Geometry check sheet. Reference: the model listing, model coordinates, mm. A direction names the side the tool comes from. Round coordinates to 2 decimals unless told otherwise and drop trailing zeros. Write each loop counter-clockwise with the first axis right and the second up, starting at its lowest first coordinate (ties: lowest second). Pieces come first, ordered by that corner, then holes. Notation, with made-up numbers: M -3,10.5 L 30,10.5 A13 ccw 30,34.5 Z; hole C 24,3 d7. An arc over 180 degrees is marked long. Put each result on its own line as item: value. Start each with the question number.
(1) Section check C-C on z = 31. Record the cut outline in (x, y).
(2) Tool access check on faces 1 (the cylindrical face through (-15.88, 54.97, 17.32)), 2 (the cylindrical face through (7.086, 50.465, -17.089)), 3 (the flat face through (19.04, 24, 10.33)). Record the directions out of +Z, -Z, +X, -X, +Y, -Y that give a thin tool (end or side, any length) a straight path to the whole face; none if there is none.
(3) Section check D-D on x = 35.5. Record the cut outline in (y, z).
(4) Gauge pin test, flat ends, axial feed: pin 1 (3 mm diameter, centred on y = 49, z = -12.5, fed in from +X); pin 2 (1 mm diameter, centred on y = 16.5, z = 21.5, fed in from +X); pin 3 (10 mm diameter, centred on x = -16.5, y = 57.5, fed in from +Z); pin 4 (1 mm diameter, centred on x = 21, z = 13, fed in from -Y). Record the tip position at first contact, or that the pin passes through.
(5) Material ranges on probe 1 along X at (y, z) = (49.95, 0); probe 2 along Z at (x, y) = (1, 39.5); probe 3 along X at (y, z) = (38.75, 0), recorded low to high.
from build123d import *


with BuildPart() as part:
    # 草图1 → 旋转1 (revolve)
    with BuildSketch(Plane.XY, mode=Mode.PRIVATE) as revolve_1_sk:
        Polygon((-23.5, 57), (-23.5, 53), (-18.5, 53), (-18.5, 48), (-21.5, 48), (-21.5, 24), (-23.5, 24), (-23.5, 0), (-41.5, 0), (-41.5, 6), (-29.5, 6), (-29.5, 20), (-28.5, 20), (-28.5, 67), (-24.5, 67), (-24.5, 57), align=None)
    revolve(revolve_1_sk.sketch.rotate(Axis((0, 0, 0), (0, 1, 0)), 270), axis=Axis((0, 0, 0), (0, 1, 0)))


solid = part.part
Answers follow:
1. outline: M -27.59,0 L 27.59,0 L 27.59,6 L -27.59,6 Z
2. face 1: +Y
2. face 2: +Y, -Y
2. face 3: -Y
3. outline: M 0,-21.49 L 6,-21.49 L 6,21.49 L 0,21.49 Z
4. pin 1: stops at x = 26.29
4. pin 2: stops at x = 20.72
4. pin 3: stops at z = 26.08
4. pin 4: stops at y = 0
5. probe 1: x = -28.5 to -18.5, 18.5 to 28.5
5. probe 2: z = -28.48 to -21.48, 21.48 to 28.48
5. probe 3: x = -28.5 to -21.5, 21.5 to 28.5
